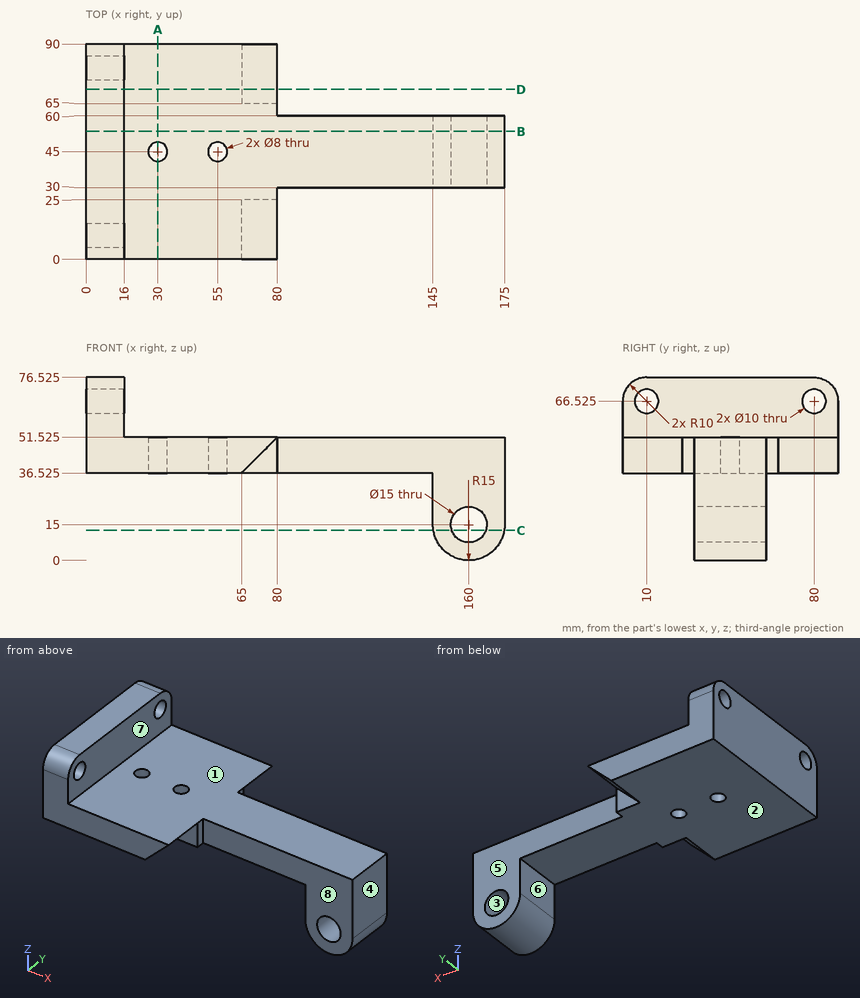
Here's the drawing with two shaded views (mm, measured from the low corner). I have some questions. A direction names the side the tool comes from. Give positions to 0.01 mm unless a question says otherwise; leave off trailing zeros. Loops run counter-clockwise (first coordinate to the right, second up) from the corner with the lowest first, then second, coordinate; pieces in that order, holes last. Notation, with made-up numbers: M 58,67.25 L 76,67.25 A22 cw 76,74.25 Z; hole C -13,70 d6. An arc over 180 degrees is marked long. One line per item, written item: value.
1) Please list where these lines run through material, in increasing order: line 1 (X direction, y = 45, z = 48.25); line 2 (Y direction, x = 55, z = 45); line 3 (X direction, y = 38, z = 15).
Geometry check:
line 1: x = 0 to 26, 34 to 51, 59 to 175
line 2: y = 0 to 41, 49 to 90
line 3: x = 145 to 152.5, 167.5 to 175
2) Thinking about a two-plate mould opening in Z: for the marked faces 1, 2, 3 and 4, which applies, +Z half, -Z half, draft (parallel to the pull), parting line (faces both ways), or undercut?
Geometry check:
face 1: +Z half
face 2: -Z half
face 3: undercut
face 4: draft
3) Imagine slicing it at A-A on x = 30. Write out the boundary of the cut face in (y, z) (3 decimals), and give its area (3 significant figures).
Geometry check:
outline: M 0,36.525 L 41,36.525 L 41,51.525 L 0,51.525 Z; M 49,36.525 L 90,36.525 L 90,51.525 L 49,51.525 Z
area: 1,230 mm²
4) Imagine slicing it at D-D on y = 71. Write out the boundary of the cut face in (x, z) (3 decimals).
Geometry check:
outline: M 0,36.525 L 65,36.525 L 80,51.525 L 16,51.525 L 16,76.525 L 0,76.525 Z
5) On a 3-axis mill with a long thin cutter (end or side, diameter ignored), from which of +Z, -Z, +X, -X, +Y, -Y can I reach the whole of each face in a straight line? I mean the marked faces 5, 6, 7 and 8. Say none if no direction works.
Geometry check:
face 5: +Z, -Z, +X, +Y
face 6: -Z, -X, +Y, -Y
face 7: +Z, +X, +Y, -Y
face 8: +Z, -Z, +X, -Y
6) I'm going to push flat-ended pins straight in: pin 1 (10 mm diameter, centred on y = 47.5, z = 58, fed in from +X); pin 2 (10.5 mm diameter, centred on x = 55, y = 45, fed in from -Z) (3 decimals); pin 3 (1.5 mm diameter, centred on y = 61.5, z = 47.5, fed in from +X). Where does each tip first touch, or does it pass through?
Geometry check:
pin 1: stops at x = 16
pin 2: stops at z = 36.525
pin 3: stops at x = 80
7) Imagine slicing it at C-C on z = 12.5. Write out the boundary of the cut face in (x, y).
Geometry check:
outline: M 145.21,30 L 152.93,30 L 152.93,60 L 145.21,60 Z; M 167.07,30 L 174.79,30 L 174.79,60 L 167.07,60 Z
8) Imagine slicing it at B-B on y = 53.5. Write out the boundary of the cut face in (x, z) (3 decimals).
Geometry check:
outline: M 0,36.525 L 145,36.525 L 145,15 A15 ccw 175,15 L 175,51.525 L 16,51.525 L 16,76.525 L 0,76.525 Z; hole C 160,15 d15
